```python
from build123d import *

# Parameters (mm, degrees)
EXTRUDE_1_DEPTH     = 15
HOLE_WIZARD_M20_1_D = 17.5


with BuildPart() as part:
    # 草图1 → 凸台-拉伸1 (new body)
    with BuildSketch(Plane(origin=(0, 0, 0), x_dir=(1, 0, 0), z_dir=(0, 1, 0))):
        Polygon((0, 17.320508076), (-15, 8.660254038), (-15, -8.660254038), (0, -17.320508076), (15, -8.660254038), (15, 8.660254038), align=None)
    extrude(amount=EXTRUDE_1_DEPTH)

    # M20 螺纹孔1 (through all)
    with Locations(Plane(origin=(0, 15, 0), x_dir=(1, 0, 0), z_dir=(0, 1, 0))):
        with Locations((0, 0)):
            Hole(HOLE_WIZARD_M20_1_D / 2)


solid = part.part
```
Design review of the part built by this model. Coordinates are the model's own, in mm. Give positions to 0.01 mm unless a question says otherwise; leave off trailing zeros. Order: outer loops, then holes, each group sorted by start corner. A loop starts at its lowest first (then second) coordinate and runs counter-clockwise, first axis right, second up. Notation, with made-up numbers: (46.25, 7) -> (51.25, 7) arc R30 ccw to (51.25, 44) -> close; hole circle Ø11 at (73.5, 51). An arc over 180 degrees is marked (long way). Write each question's results on one line, items separated by ' | '. Start each with the question number.
Q1. Add section B-B on y = 2. Give the boundary of the cut face in (x, z).
Q2. Add section C-C on x = -1. Give the boundary of the cut face in (y, z).
Q3. Mouldability with a two-part tool opening along Z and no side actions: class faces 1 (the cylindrical face through (6.944, 7.395, 5.324)), 2 (the flat face through (15, 7, 0)), 3 (the flat face through (7.605, 7.395, -12.93)), 4 (the flat face through (7.4, 7.4, 13.05)) as +Z half, -Z half, draft (parallel to the pull), parting line (faces both ways), or undercut.
Q4. Add section A-A on z = 0. Give the boundary of the cut face in (x, y), and give its area (4 significant figures).
Q5. Add section D-D on z = -15. Give the boundary of the cut face in (x, y), and give its area (3 significant figures).
Q6. Wall thickness on L1, parallel to Z at x = 0, y = 11.25; L2, parallel to Z at x = -4, y = 5.5; L3, parallel to Z at x = -9.5, y = 8.75: over which ranges is each line inside the solid? List them lowest first. Write a range as from..to.
Q7. For pin 1 (3 mm diameter, centred on y = 12.5, z = 11.5, fed in from +X); pin 2 (16 mm diameter, centred on x = 0, z = 0, fed in from -Y); pin 3 (4 mm diameter, centred on y = 9, z = -10, fed in from -X); pin 4 (1 mm diameter, centred on x = 5.5, y = 2.5, fed in from +Z), all flat-tipped, find the tip position at first contact; note any pin that passes through.
Found:
1) outline: (-15, -8.66) -> (0, -17.32) -> (15, -8.66) -> (15, 8.66) -> (0, 17.32) -> (-15, 8.66) -> close; hole circle Ø17.5 at (0, 0)
2) outline: (0, -16.74) -> (15, -16.74) -> (15, -8.69) -> (0, -8.69) -> close; (0, 8.69) -> (15, 8.69) -> (15, 16.74) -> (0, 16.74) -> close
3) face 1: undercut | face 2: draft | face 3: -Z half | face 4: +Z half
4) outline: (-15, 0) -> (-8.75, 0) -> (-8.75, 15) -> (-15, 15) -> close; (8.75, 0) -> (15, 0) -> (15, 15) -> (8.75, 15) -> close | area: 187.5 mm2
5) outline: (-4.02, 0) -> (4.02, 0) -> (4.02, 15) -> (-4.02, 15) -> close | area: 121 mm2
6) L1: z = -17.32..-8.75, 8.75..17.32 | L2: z = -15.01..-7.78, 7.78..15.01 | L3: z = -11.84..11.84
7) pin 1: stops at x = 12.68 | pin 2: passes through | pin 3: stops at x = -15 | pin 4: stops at z = 14.43
